The drawing under review shows one solid part. Ordinate dimensions are in mm from its lowest x, y, z. A direction names the side the tool comes from. Give positions to 0.01 mm unless a question says otherwise; leave off trailing zeros. Loops run counter-clockwise (first coordinate to the right, second up) from the corner with the lowest first, then second, coordinate; pieces in that order, holes last. Notation, with made-up numbers: M 37.5,27.5 L 82.5,27.5 A30 ccw 82.5,57.5 Z; hole C 30.25,21 d7. An arc over 180 degrees is marked long. One line per item, written item: value. Start each with the question number.
Q1. For the marked faces 4 and 5, list the 3-axis set-ups (+Z, -Z, +X, -X, +Y, -Y) from which the entire face can be reached by the end or side of a thin tool; tool diameter is ignored.
Q2. Mouldability with a two-part tool opening along Y and no side actions: class the marked faces 1, 2 and 3 as released by +Y, released by -Y, zero draft, split by the parting line, or undercut.
Q3. We need section C-C on x = 34. Write out the cut boundary in (y, z), plus the area to 3 significant figures.
Q4. We need section A-A on z = 13. Write out the cut boundary in (x, y), plus the area to 3 significant figures.
Q5. We need section B-B on y = 168.5. Write out the cut boundary in (x, z).
Q6. To check wall thickness, follow line 1 along Y through (x, z) = (109, 41); line 2 along X through (y, z) = (63, 35); line 3 along Z through (x, y) = (43, 59). State the ranges of each line that lie inside material, in increasing order. Write a range as from..to.
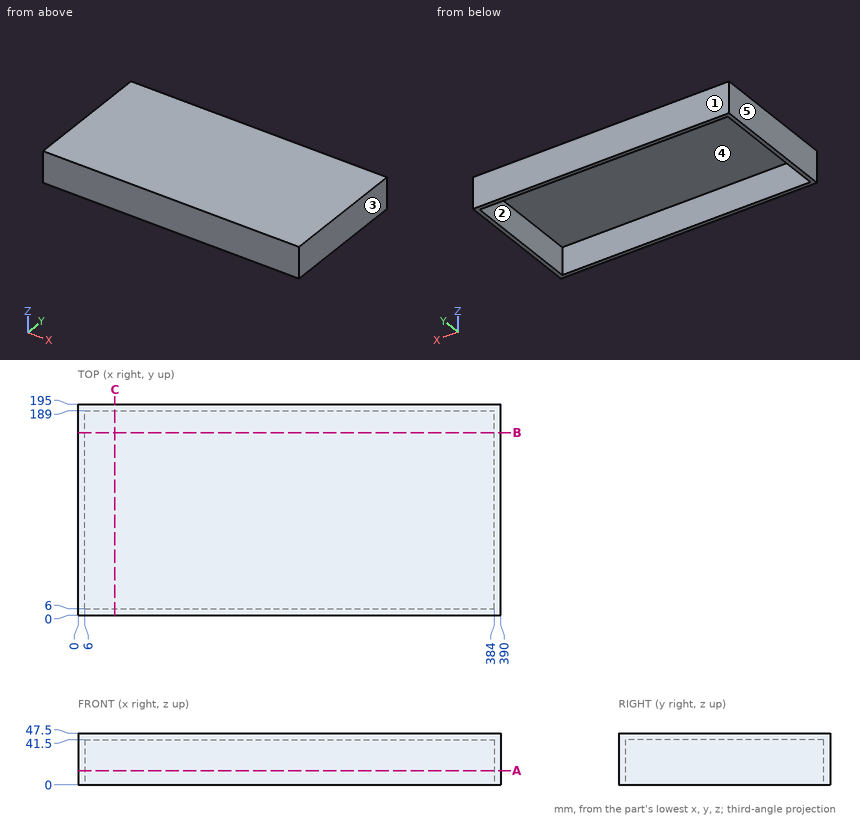
Solved:
1. face 4: -Z
1. face 5: +Z, -Z, -X, +Y, -Y
2. face 1: released by +Y
2. face 2: undercut
2. face 3: zero draft
3. outline: M 0,0 L 6,0 L 6,41.5 L 189,41.5 L 189,0 L 195,0 L 195,47.5 L 0,47.5 Z
3. area: 1,670 mm2
4. outline: M 0,0 L 390,0 L 390,195 L 0,195 Z; hole M 6,6 L 384,6 L 384,189 L 6,189 Z
4. area: 6,880 mm2
5. outline: M 0,0 L 6,0 L 6,41.5 L 384,41.5 L 384,0 L 390,0 L 390,47.5 L 0,47.5 Z
6. line 1: 0..6, 189..195
6. line 2: 0..6, 384..390
6. line 3: 41.5..47.5
